Can you work these out from the drawing? Everything is in mm from the part's minimum corner. Give positions to 0.01 mm unless a question says otherwise; leave off trailing zeros. Order: outer loops, then holes, each group sorted by start corner. A loop starts at its lowest first (then second) coordinate and runs counter-clockwise, first axis right, second up. Notation, with made-up numbers: M -13,-30 L 36,-30 A14 ccw 36,-6 Z; hole C -30,65.5 d3. An arc over 180 degrees is marked long. Use a Markdown table: item, result. Add a question column.
Item 1: Suppose I cut it at A-A on x = 110. Write out the boundary of the cut face in (y, z).
Item 2: Suppose I cut it at C-C on z = 7.5. Write out the boundary of the cut face in (x, y).
Item 3: Suppose I cut it at D-D on x = 186.5. Write out the boundary of the cut face in (y, z).
Item 4: If I drill on L1, parallel to Y at x = 110, z = 8; L2, parallel to Y at x = 101.5, z = 2.5; L3, parallel to Y at x = 208, z = 9.5, over which ranges is the centre line in solid material (lowest first)? Write a range as from..to.
Item 5: I'm going to push flat-ended pins straight in: pin 1 Ø4 at (y, z) = (52, 8.5) entering from +X; pin 2 Ø1.5 at (x, z) = (54, 2.5) entering from -Y; pin 3 Ø15 at (x, y) = (110, 180) entering from -Z; pin 4 Ø3 at (y, z) = (40, 6) entering from +X. Where does each tip first touch, or does it pass through?
Item 6: Suppose I cut it at B-B on y = 180. Write out the boundary of the cut face in (x, z), plus the area to 3 significant figures.
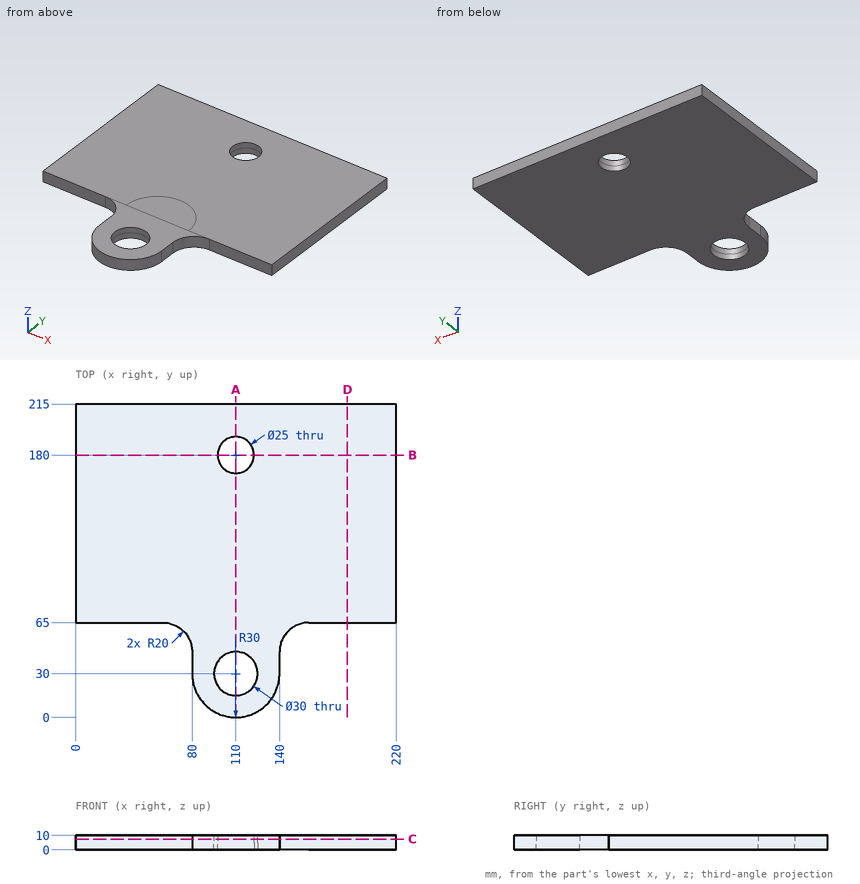
Findings below:
| question | item | result |
|---|---|---|
| 1 | outline | M 0,0 L 15,0 L 15,10 L 0,10 Z; M 45,0 L 167.5,0 L 167.5,10 L 45,10 Z; M 192.5,0 L 215,0 L 215,10 L 192.5,10 Z |
| 2 | outline | M 0,65 L 60,65 A20 cw 80,45 L 80,30 A30 ccw 140,30 L 140,45 A20 cw 160,65 L 220,65 L 220,215 L 0,215 Z; hole C 110,30 d30; hole C 110,180 d25 |
| 3 | outline | M 65,0 L 215,0 L 215,10 L 65,10 Z |
| 4 | L1 | y = 0..15, 45..167.5, 192.5..215 |
| 4 | L2 | y = 1.23..17.64, 42.36..170.83, 189.17..215 |
| 4 | L3 | y = 65..215 |
| 5 | pin 1 | stops at x = 142.14 |
| 5 | pin 2 | stops at y = 65 |
| 5 | pin 3 | passes through |
| 5 | pin 4 | stops at x = 140 |
| 6 | outline | M 0,0 L 97.5,0 L 97.5,10 L 0,10 Z; M 122.5,0 L 220,0 L 220,10 L 122.5,10 Z |
| 6 | area | 1,950 mm^2 |
